Check sheet for the modelled part. Datum: model origin and axes. Units: mm. Face numbers are marked on the shaded views. Round coordinates to 2 decimals unless told otherwise and drop trailing zeros. Order: outer loops, then holes, each group sorted by start corner. A loop starts at its lowest first (then second) coordinate and runs counter-clockwise, first axis right, second up. Notation, with made-up numbers: (24, -36) -> (75, -36) arc R17 ccw to (75, -9) -> close; hole circle Ø8 at (32.5, -9). An arc over 180 degrees is marked (long way). Answer in a Markdown table with one row per item.
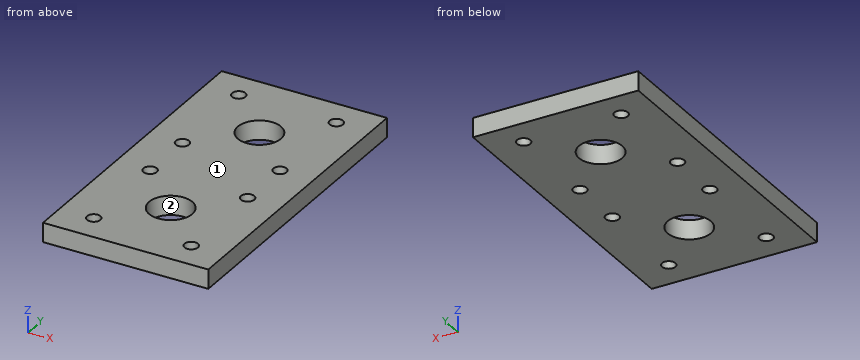
from build123d import *

# Parameters (mm, degrees)
SKETCH_1_W          = 172
SKETCH_1_H          = 322
EXTRUDE_1_DEPTH     = 20
SKETCH_3_R          = 22.5
SKETCH_3_R_2        = 7
CUT_EXTRUDE_1_DEPTH = 184.621894119


with BuildPart() as part:
    # 草图1 → 凸台-拉伸1 (new body)
    with BuildSketch(Plane.XY):
        Rectangle(SKETCH_1_W, SKETCH_1_H)
    extrude(amount=EXTRUDE_1_DEPTH)

    # 草图3 → 切除-拉伸1 (cut, through all)
    with BuildSketch(Plane(origin=(0, 0, 0), x_dir=(-1, 0, 0), z_dir=(0, 0, -1))):
        with Locations((0, 80)):
            Circle(SKETCH_3_R)
        with Locations((-50.75, 130.75)):
            Circle(SKETCH_3_R_2)
        with Locations((50.75, 130.75)):
            Circle(SKETCH_3_R_2)
        with Locations((-50.75, 29.25)):
            Circle(SKETCH_3_R_2)
        with Locations((50.75, 29.25)):
            Circle(SKETCH_3_R_2)
        with Locations((0, -79.81)):
            Circle(SKETCH_3_R)
        with Locations((-50.75, -29.06)):
            Circle(SKETCH_3_R_2)
        with Locations((50.75, -29.06)):
            Circle(SKETCH_3_R_2)
        with Locations((50.75, -130.56)):
            Circle(SKETCH_3_R_2)
        with Locations((-50.75, -130.56)):
            Circle(SKETCH_3_R_2)
    extrude(amount=-CUT_EXTRUDE_1_DEPTH, mode=Mode.SUBTRACT)


solid = part.part
Item 1: Cross-section at B-B (x = -50.75). Record the boundary of the cut face in (y, z).
Result sheet:
| item | result |
|---|---|
| outline | (-161, 0) -> (-137.56, 0) -> (-137.56, 20) -> (-161, 20) -> close; (-123.56, 0) -> (-36.06, 0) -> (-36.06, 20) -> (-123.56, 20) -> close; (-22.06, 0) -> (22.25, 0) -> (22.25, 20) -> (-22.06, 20) -> close; (36.25, 0) -> (123.75, 0) -> (123.75, 20) -> (36.25, 20) -> close; (137.75, 0) -> (161, 0) -> (161, 20) -> (137.75, 20) -> close |
Item 2: Mould release check, pull along X, two halves, no side actions. Record for the marked faces 1 and 2: pulls with the +X half, pulls with the -X half, needs draft (parallel to the pull), parting line crosses it, or undercut.
Result sheet:
| item | result |
|---|---|
| face 1 | needs draft |
| face 2 | undercut |
Item 3: Cross-section at A-A (y = 29.25). Record the boundary of the cut face in (x, z), and give its area (3 significant figures).
Result sheet:
| item | result |
|---|---|
| outline | (-86, 0) -> (-57.75, 0) -> (-57.75, 20) -> (-86, 20) -> close; (-43.75, 0) -> (43.75, 0) -> (43.75, 20) -> (-43.75, 20) -> close; (57.75, 0) -> (86, 0) -> (86, 20) -> (57.75, 20) -> close |
| area | 2,880 mm^2 |
Item 4: Scan lines: line 1 (Y direction, x = -50.75, z = 9.75); line 2 (Y direction, x = 5, z = 2.25); line 3 (Y direction, x = -17.5, z = 3). Record each from-to range of solid material in increasing order. Write a range as [from, to].
Result sheet:
| item | result |
|---|---|
| line 1 | y = [-161, -137.56], [-123.56, -36.06], [-22.06, 22.25], [36.25, 123.75], [137.75, 161] |
| line 2 | y = [-161, -101.75], [-57.87, 58.06], [101.94, 161] |
| line 3 | y = [-161, -93.95], [-65.67, 65.86], [94.14, 161] |
Item 5: Cross-section at D-D (y = -79.81). Record the boundary of the cut face in (x, z).
Result sheet:
| item | result |
|---|---|
| outline | (-86, 0) -> (-22.5, 0) -> (-22.5, 20) -> (-86, 20) -> close; (22.5, 0) -> (86, 0) -> (86, 20) -> (22.5, 20) -> close |
Item 6: Cross-section at C-C (x = 0). Record the boundary of the cut face in (y, z), and give its area (3 significant figures).
Result sheet:
| item | result |
|---|---|
| outline | (-161, 0) -> (-102.31, 0) -> (-102.31, 20) -> (-161, 20) -> close; (-57.31, 0) -> (57.5, 0) -> (57.5, 20) -> (-57.31, 20) -> close; (102.5, 0) -> (161, 0) -> (161, 20) -> (102.5, 20) -> close |
| area | 4,640 mm^2 |
Item 7: Depth check by flat-ended pin: P1, Ø11, axis at x = -50.75, y = -29.06, coming from the +Z side. Enter the tip coordinate at first touch or a pass-through.
Result sheet:
| item | result |
|---|---|
| P1 | passes through |
